```python
from build123d import *

# Parameters (mm, degrees)
SKETCH_1_R      = 10
SKETCH_1_R_2    = 7.55
EXTRUDE_1_DEPTH = 2
CHAMFER_1_SIZE  = 0.2


with BuildPart() as part:
    # 草图1 → 凸台-拉伸1 (new body)
    with BuildSketch(Plane(origin=(0, 0, 0), x_dir=(0, 0, -1), z_dir=(1, 0, 0))):
        Circle(SKETCH_1_R)
        Circle(SKETCH_1_R_2, mode=Mode.SUBTRACT)
    extrude(amount=EXTRUDE_1_DEPTH)

    # 倒角1
    chamfer_1_edges = [part.edges().sort_by_distance(p)[0] for p in [
        (0, 0, 10),
        (2, 0, 10),
        (0, 0, 7.55),
        (2, 0, 7.55),
    ]]
    chamfer(chamfer_1_edges, length=CHAMFER_1_SIZE)


solid = part.part
```
Can you work these out from the model? Positions are in its coordinate system, mm. Coordinates: 2 decimals unless noted, no trailing zeros. Order: outer loops, then holes, each group sorted by start corner. A loop starts at its lowest first (then second) coordinate and runs counter-clockwise, first axis right, second up. Notation, with made-up numbers: (11.25, 49) - (17.25, 49) arc R26 cw to (17.25, 87) - close; hole circle Ø3 at (72.25, 13). An arc over 180 degrees is marked (long way). Answer in a Markdown table with one row per item.
1. If we mould it in two halves opening along Z, with no side actions, what happens to faces 1 (the cylindrical face through (0.99, -9.76, 2.17)), 2 (the cylindrical face through (0.99, -7.37, 1.64)), 3 (the flat face through (0, 8, -1))? For each: pulls with the +Z half, pulls with the -Z half, needs draft (parallel to the pull), parting line crosses it, or undercut.
Reply:
| item | result |
|---|---|
| face 1 | parting line crosses it |
| face 2 | undercut |
| face 3 | needs draft |
2. Suppose I cut it at A-A (z = 0). Please give me the cut outline in (x, y).
Reply:
| item | result |
|---|---|
| outline | (0, -9.8) - (0.2, -10) - (1.8, -10) - (2, -9.8) - (2, -7.75) - (1.8, -7.55) - (0.2, -7.55) - (0, -7.75) - close; (0, 7.75) - (0.2, 7.55) - (1.8, 7.55) - (2, 7.75) - (2, 9.8) - (1.8, 10) - (0.2, 10) - (0, 9.8) - close |
3. If I drill on line 1 along Y through (x, z) = (1.45, 0); line 2 along Y through (x, z) = (0.3, 4.5); line 3 along Z through (x, y) = (1.75, 1.25), over which ranges is the centre line in solid material (lowest first)?
Reply:
| item | result |
|---|---|
| line 1 | y = -10 to -7.55, 7.55 to 10 |
| line 2 | y = -8.93 to -6.06, 6.06 to 8.93 |
| line 3 | z = -9.92 to -7.45, 7.45 to 9.92 |
4. Suppose I cut it at C-C (x = 0.7). Please give me the cut outline in (y, z).
Reply:
| item | result |
|---|---|
| outline | circle Ø20 at (0, 0); hole circle Ø15.1 at (0, 0) |
5. For pin 1 (9 mm diameter, centred on y = 0, z = 0, fed in from -X), with a flat end and sliding along its axis, tell me the tip position at first contact or that it passes through.
Reply:
| item | result |
|---|---|
| pin 1 | passes through |
